from build123d import *

# Parameters (mm, degrees)
BRACKET_BODY_DEPTH        = 27
CLAMP_SLOT_DEPTH          = 54
CLAMP_END_TRIM_DEPTH      = 54
MOUNTING_HOLES_SKETCH_R   = 3.5
MOUNTING_HOLES_6X_7_DEPTH = 54


with BuildPart() as part:
    # Bracket Profile Sketch → Bracket Body (new, symmetric)
    with BuildSketch(Plane.XY):
        Polygon((108.258330249, 16.016660498), (99.258330249, 0.42820323), (86.143593539, 8), (0, 8), (0, 0), (84, 0), (140.291651246, -32.5), (153.291651246, -9.983339502), align=None)
    extrude(amount=BRACKET_BODY_DEPTH, both=True)

    # Clamp Slot Sketch → Clamp Slot (cut)
    with BuildSketch(Plane(origin=(119.291651246, -68.873066959, 0), x_dir=(0, 0, -1), z_dir=(0.8660254037844386, -0.5000000000000001, 0))):
        Polygon((-17.5, 50), (17.5, 50), (17.5, 58), (5, 58), (5, 68), (-5, 68), (-5, 58), (-17.5, 58), align=None)
    extrude(amount=-CLAMP_SLOT_DEPTH, mode=Mode.SUBTRACT)

    # Clamp End Trim Sketch → Clamp End Trim (cut)
    with BuildSketch(Plane(origin=(34, 58.889727457, 0), x_dir=(0.8660254037844384, -0.5000000000000007, 0), z_dir=(0.5000000000000006, 0.8660254037844383, 0))):
        with BuildLine():
            Line((130.187106004, 27), (186.710578253, 27))
            Line((186.710578253, 27), (186.710578253, -27))
            Line((186.710578253, -27), (130.187106004, -27))
            ThreePointArc((130.187106004, -27), (137.746133918, 0), (130.187106004, 27))
        make_face()
    extrude(amount=-CLAMP_END_TRIM_DEPTH, mode=Mode.SUBTRACT)

    # Mounting Holes Sketch → Mounting Holes 6xØ7 (cut)
    with BuildSketch(Plane(origin=(0, 8, 0), x_dir=(1, 0, 0), z_dir=(0, 1, 0))):
        with Locations(Location((11, 16, 0), (0, 0, 270))):
            Circle(MOUNTING_HOLES_SKETCH_R)
        with Locations(Location((43, 16, 0), (0, 0, 270))):
            Circle(MOUNTING_HOLES_SKETCH_R)
        with Locations(Location((75, 16, 0), (0, 0, 270))):
            Circle(MOUNTING_HOLES_SKETCH_R)
        with Locations(Location((11, -16, 0), (0, 0, 270))):
            Circle(MOUNTING_HOLES_SKETCH_R)
        with Locations(Location((43, -16, 0), (0, 0, 270))):
            Circle(MOUNTING_HOLES_SKETCH_R)
        with Locations(Location((75, -16, 0), (0, 0, 270))):
            Circle(MOUNTING_HOLES_SKETCH_R)
    extrude(amount=-MOUNTING_HOLES_6X_7_DEPTH, mode=Mode.SUBTRACT)


solid = part.part
The model under review builds one solid part; all positions refer to its coordinate system, in mm. A direction names the side the tool comes from. Round coordinates to 2 decimals unless told otherwise and drop trailing zeros. Loops run counter-clockwise (first coordinate to the right, second up) from the corner with the lowest first, then second, coordinate; pieces in that order, holes last. Notation, with made-up numbers: (38.5, 47.25) -> (91.5, 47.25) arc R20 cw to (91.5, 56.25) -> close; hole circle Ø9 at (35.5, 16). An arc over 180 degrees is marked (long way). Return JSON: item names as keys, results as strings.
(1) For pin 1 (1.5 mm diameter, centred on y = 9.5, z = 3.5, fed in from +X); pin 2 (6 mm diameter, centred on y = -3.5, z = 17, fed in from +X); pin 3 (9 mm diameter, centred on x = 11, z = 16, fed in from +Y); pin 4 (1.5 mm diameter, centred on x = 35.5, z = 19.5, fed in from -Y), all flat-tipped, find the tip position at first contact; note any pin that passes through.
Solved:
{"pin 1": "through", "pin 2": "x = 147.26", "pin 3": "y = 8", "pin 4": "y = 0"}
(2) Add section A-A on x = 43. Write out the cut boundary in (y, z), plus the area to 3 significant figures.
Solved:
{"outline": "(0, -27) -> (8, -27) -> (8, -19.5) -> (0, -19.5) -> close; (0, -12.5) -> (8, -12.5) -> (8, 12.5) -> (0, 12.5) -> close; (0, 19.5) -> (8, 19.5) -> (8, 27) -> (0, 27) -> close", "area": "320 mm2"}
(3) The part is to be moulded in two halves that separate along Z. For faces 1 (the cylindrical face through (71.895, 4.056, 17.615)), 2 (the flat face through (104.82, 10.06, -18.29)), 3 (the flat face through (89, 0, -27)), 4 (the flat face through (125.98, -5.76, 11.16)), say which applies: released by +Z, released by -Z, zero draft, split by the parting line, or undercut.
Solved:
{"face 1": "undercut", "face 2": "zero draft", "face 3": "released by -Z", "face 4": "undercut"}
(4) For line 1 (X direction, y = 3.75, z = -16); line 2 (X direction, y = 4.5, z = 16); line 3 (Z direction, x = 40.5, y = 0.5), list the stretches that pass through material, from the lowest coordinate up.
Solved:
{"line 1": "0 to 7.5, 14.5 to 39.5, 46.5 to 71.5, 78.5 to 93.5, 109.5 to 129.5", "line 2": "0 to 7.5, 14.5 to 39.5, 46.5 to 71.5, 78.5 to 92.21, 108.21 to 128.21", "line 3": "-27 to -18.45, -13.55 to 13.55, 18.45 to 27"}
(5) For faces 5 (the flat face through (44, 8, 0)), 6 (the flat face through (0, 4, 0)), 7 (the flat face through (123, -8, 17.5)), 8 (the flat face through (104.82, 10.06, 18.6)), 9 (the flat face through (128, -1, -5)), list the 3-axis set-ups (+Z, -Z, +X, -X, +Y, -Y) from which the entire face can be reached by the end or side of a thin tool; tool diameter is ignored.
Solved:
{"face 5": "+Z, -Z, -X, +Y", "face 6": "+Z, -Z, -X, +Y, -Y", "face 7": "none", "face 8": "+Z, -Z, +Y", "face 9": "+X, +Y"}
(6) Add section D-D on y = 12. Write out the cut boundary in (x, z), plus the area to 3 significant figures.
Solved:
{"outline": "(105.94, -27) -> (115.22, -27) -> (115.22, -5) -> (105.94, -5) -> close; (105.94, 5) -> (115.22, 5) -> (115.22, 27) -> (105.94, 27) -> close", "area": "408 mm2"}
(7) Add section C-C on z = -16. Write out the cut boundary in (x, y), plus the area to 3 significant figures.
Solved:
{"outline": "(0, 0) -> (7.5, 0) -> (7.5, 8) -> (0, 8) -> close; (14.5, 0) -> (39.5, 0) -> (39.5, 8) -> (14.5, 8) -> close; (46.5, 0) -> (71.5, 0) -> (71.5, 8) -> (46.5, 8) -> close; (78.5, 0) -> (84, 0) -> (138.11, -31.24) -> (142.11, -24.31) -> (86.14, 8) -> (78.5, 8) -> close; (103.26, 7.36) -> (146.11, -17.38) -> (151.11, -8.72) -> (108.26, 16.02) -> close", "area": "1,520 mm2"}
(8) Add section B-B on y = 5. State how many separate pieces and enclosed holes the cut face has, plus the area to 3 significant figures.
Solved:
{"separate pieces": "3", "enclosed holes": "6", "area": "5,680 mm2"}
